The listing builds one solid part. Answer for the finished solid, in the listing's coordinates (mm). A direction names the side the tool comes from. Coordinates: 2 decimals unless noted, no trailing zeros. Use one line per item in the form item = value. Start each with the question number.
Item 1: A tool of negligible diameter and unlimited length cuts with its end or side. For faces 4 (the flat face through (340, 14, 0)), 5 (the flat face through (340, 20, 11)), from which of +Z, -Z, +X, -X, +Y, -Y can it reach the whole face along a straight path? Write none if from no direction.
Item 2: Consider line 1 along Z through (x, y) = (521, -4); line 2 along Z through (x, y) = (640, -11). Determine where each line is inside the solid, lowest interval first. Write a range as [from, to].
Item 3: The mould has two halves that part along Y. Classify faces 1 (the flat face through (340, 0, 14)), 2 (the flat face through (340, -20, -11)), 3 (the flat face through (340, -12, -20)): released by +Y, released by -Y, zero draft, split by the parting line, or undercut.
from build123d import *

# Parameters (mm, degrees)
SKETCH1_W           = 26
SKETCH1_H           = 26
BOSS_EXTRUDE1_DEPTH = 690


with BuildPart() as part:
    # Sketch1 → Boss-Extrude1 (new body)
    with BuildSketch(Plane(origin=(0, 0, 0), x_dir=(0, 0, -1), z_dir=(1, 0, 0))):
        Polygon((-20, -20), (-3, -20), (-3, -17), (-6.5, -17), (-6.5, -14), (6.5, -14), (6.5, -17), (3, -17), (3, -20), (20, -20), (20, -3), (17, -3), (17, -6.5), (14, -6.5), (14, 6.5), (17, 6.5), (17, 3), (20, 3), (20, 20), (3, 20), (3, 17), (6.5, 17), (6.5, 14), (-6.5, 14), (-6.5, 17), (-3, 17), (-3, 20), (-20, 20), (-20, 3), (-17, 3), (-17, 6.5), (-14, 6.5), (-14, -6.5), (-17, -6.5), (-17, -3), (-20, -3), align=None)
        Rectangle(SKETCH1_W, SKETCH1_H, mode=Mode.SUBTRACT)
    extrude(amount=BOSS_EXTRUDE1_DEPTH)


solid = part.part
Response:
q1.face_4 = +X, -X
q1.face_5 = +Z, -Z, +X, -X, +Y
q2.line_1 = [-20, -17], [-14, -13], [13, 14], [17, 20]
q2.line_2 = [-20, -13], [13, 20]
q3.face_1 = undercut
q3.face_2 = released by -Y
q3.face_3 = zero draft
